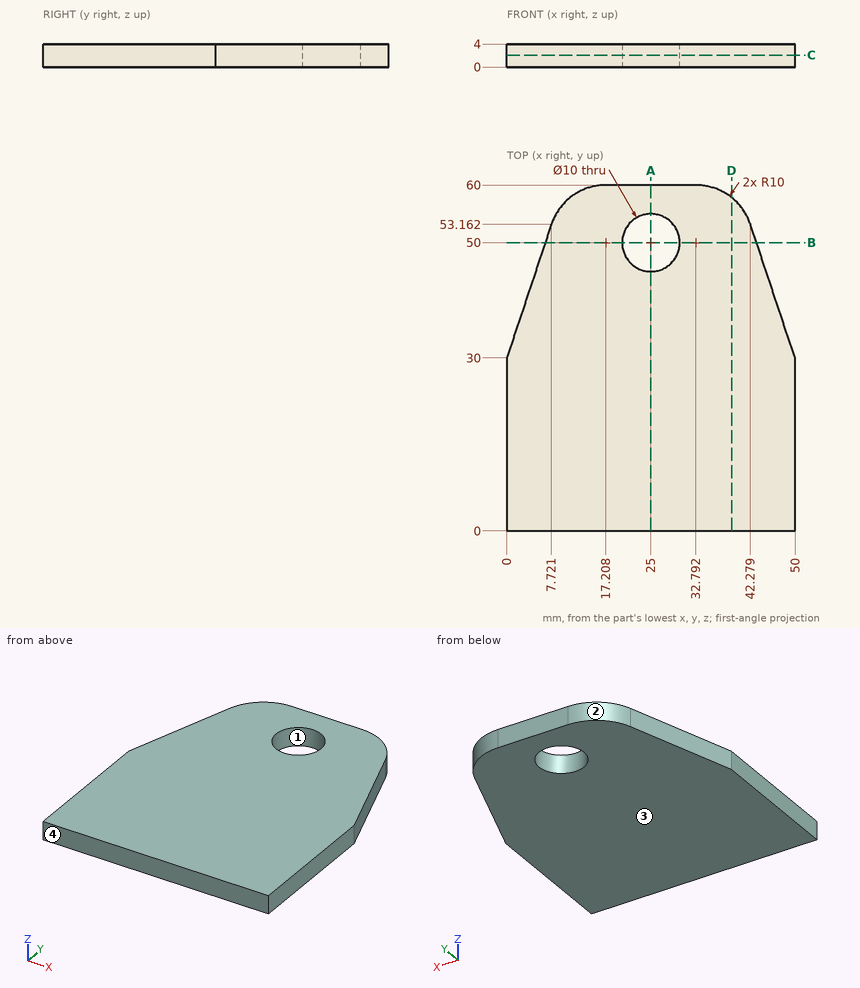
Design review of the part shown in the three views and the two pictorial views. Dimensions are in mm from the part's minimum x, y and z. Give positions to 0.01 mm unless a question says otherwise; leave off trailing zeros. Order: outer loops, then holes, each group sorted by start corner. A loop starts at its lowest first (then second) coordinate and runs counter-clockwise, first axis right, second up. Notation, with made-up numbers: (84, -22.75) -> (131, -22.75) arc R19 cw to (131, 3.25) -> close; hole circle Ø9 at (38.5, 14.5). An arc over 180 degrees is marked (long way). Write each question's results on one line, items separated by ' | '. Start each with the question number.
Q1. Add section C-C on z = 2.05. Give the boundary of the cut face in (x, y), and give its area (3 significant figures).
Q2. Add section B-B on y = 50. Give the boundary of the cut face in (x, z), and give its area (3 significant figures).
Q3. Add section D-D on x = 39. Give the boundary of the cut face in (y, z).
Q4. Mouldability with a two-part tool opening along Y and no side actions: class the marked faces 1, 2, 3 and 4 as +Y half, -Y half, draft (parallel to the pull), parting line (faces both ways), or undercut.
Q5. For pin 1 (1 mm diameter, centred on y = 54, z = 0.5, fed in from -X), flat-tipped, find the tip position at first contact; note if it passes through.
Q6. Add section A-A on x = 25. Give the boundary of the cut face in (y, z).
Q7. Wall thickness on L1, parallel to Y at x = 25, z = 1.65; L2, parallel to X at y = 49.5, z = 0.4 (1 decimal); L3, parallel to X at y = 51.5, z = 1.6: over which ranges is each line inside the solid? List them lowest first. Write a range as from..to.
Found:
1) outline: (0, 0) -> (50, 0) -> (50, 30) -> (42.28, 53.16) arc R10 ccw to (32.79, 60) -> (17.21, 60) arc R10 ccw to (7.72, 53.16) -> (0, 30) -> close; hole circle Ø10 at (25, 50) | area: 2,600 mm2
2) outline: (6.67, 0) -> (20, 0) -> (20, 4) -> (6.67, 4) -> close; (30, 0) -> (43.33, 0) -> (43.33, 4) -> (30, 4) -> close | area: 107 mm2
3) outline: (0, 0) -> (57.84, 0) -> (57.84, 4) -> (0, 4) -> close
4) face 1: undercut | face 2: +Y half | face 3: draft | face 4: -Y half
5) pin 1: stops at x = 7.84
6) outline: (0, 0) -> (45, 0) -> (45, 4) -> (0, 4) -> close; (55, 0) -> (60, 0) -> (60, 4) -> (55, 4) -> close
7) L1: y = 0..45, 55..60 | L2: x = 6.5..20, 30..43.5 | L3: x = 7.17..20.23, 29.77..42.83
